from build123d import *

# Parameters (mm, degrees)
GEAR_BODY_12T_DEPTH  = 56
FACE_RECESS_SKETCH_R = 40
FACE_RECESS_80_DEPTH = 20
BORE_CUT_DEPTH       = 36


with BuildPart() as part:
    # Gear Tooth Profile Sketch → Gear Body 12T (new body)
    with BuildSketch(Plane.XY):
        with BuildLine():
            Line((-15.529142706, 57.955549577), (-17.470285544, 65.199993275))
            ThreePointArc((-17.470285544, 65.199993275), (-8.810517975, 66.922528143), (0, 67.5))
            Line((0, 67.5), (0, 60))
            ThreePointArc((0, 60), (7.831571533, 59.486691682), (15.529142706, 57.955549577))
            Line((15.529142706, 57.955549577), (17.470285544, 65.199993275))
            ThreePointArc((17.470285544, 65.199993275), (25.831131685, 62.361868445), (33.75, 58.456714755))
            Line((33.75, 58.456714755), (30, 51.961524227))
            ThreePointArc((30, 51.961524227), (36.525685741, 47.601200417), (42.426406871, 42.426406871))
            Line((42.426406871, 42.426406871), (47.72970773, 47.72970773))
            ThreePointArc((47.72970773, 47.72970773), (53.55135047, 41.091396458), (58.456714755, 33.75))
            Line((58.456714755, 33.75), (51.961524227, 30))
            ThreePointArc((51.961524227, 30), (55.432771951, 22.961005942), (57.955549577, 15.529142706))
            Line((57.955549577, 15.529142706), (65.199993275, 17.470285544))
            ThreePointArc((65.199993275, 17.470285544), (66.922528143, 8.810517975), (67.5, 0))
            Line((67.5, 0), (60, 0))
            ThreePointArc((60, 0), (59.486691682, -7.831571533), (57.955549577, -15.529142706))
            Line((57.955549577, -15.529142706), (65.199993275, -17.470285544))
            ThreePointArc((65.199993275, -17.470285544), (62.361868445, -25.831131685), (58.456714755, -33.75))
            Line((58.456714755, -33.75), (51.961524227, -30))
            ThreePointArc((51.961524227, -30), (47.601200417, -36.525685741), (42.426406871, -42.426406871))
            Line((42.426406871, -42.426406871), (47.72970773, -47.72970773))
            ThreePointArc((47.72970773, -47.72970773), (41.091396458, -53.55135047), (33.75, -58.456714755))
            Line((33.75, -58.456714755), (30, -51.961524227))
            ThreePointArc((30, -51.961524227), (22.961005942, -55.432771951), (15.529142706, -57.955549577))
            Line((15.529142706, -57.955549577), (17.470285544, -65.199993275))
            ThreePointArc((17.470285544, -65.199993275), (8.810517975, -66.922528143), (0, -67.5))
            Line((0, -67.5), (0, -60))
            ThreePointArc((0, -60), (-7.831571533, -59.486691682), (-15.529142706, -57.955549577))
            Line((-15.529142706, -57.955549577), (-17.470285544, -65.199993275))
            ThreePointArc((-17.470285544, -65.199993275), (-25.831131685, -62.361868445), (-33.75, -58.456714755))
            Line((-33.75, -58.456714755), (-30, -51.961524227))
            ThreePointArc((-30, -51.961524227), (-36.525685741, -47.601200417), (-42.426406871, -42.426406871))
            Line((-42.426406871, -42.426406871), (-47.72970773, -47.72970773))
            ThreePointArc((-47.72970773, -47.72970773), (-53.55135047, -41.091396458), (-58.456714755, -33.75))
            Line((-58.456714755, -33.75), (-51.961524227, -30))
            ThreePointArc((-51.961524227, -30), (-55.432771951, -22.961005942), (-57.955549577, -15.529142706))
            Line((-57.955549577, -15.529142706), (-65.199993275, -17.470285544))
            ThreePointArc((-65.199993275, -17.470285544), (-66.922528143, -8.810517975), (-67.5, 0))
            Line((-67.5, 0), (-60, 0))
            ThreePointArc((-60, 0), (-59.486691682, 7.831571533), (-57.955549577, 15.529142706))
            Line((-57.955549577, 15.529142706), (-65.199993275, 17.470285544))
            ThreePointArc((-65.199993275, 17.470285544), (-62.361868445, 25.831131685), (-58.456714755, 33.75))
            Line((-58.456714755, 33.75), (-51.961524227, 30))
            ThreePointArc((-51.961524227, 30), (-47.601200417, 36.525685741), (-42.426406871, 42.426406871))
            Line((-42.426406871, 42.426406871), (-47.72970773, 47.72970773))
            ThreePointArc((-47.72970773, 47.72970773), (-41.091396458, 53.55135047), (-33.75, 58.456714755))
            Line((-33.75, 58.456714755), (-30, 51.961524227))
            ThreePointArc((-30, 51.961524227), (-22.961005942, 55.432771951), (-15.529142706, 57.955549577))
        make_face()
    extrude(amount=-GEAR_BODY_12T_DEPTH)

    # Face Recess Sketch → Face Recess Ø80 (cut)
    with BuildSketch(Plane.XY):
        Circle(FACE_RECESS_SKETCH_R)
    extrude(amount=-FACE_RECESS_80_DEPTH, mode=Mode.SUBTRACT)

    # Bore Profile Sketch → Bore Cut (cut)
    with BuildSketch(Plane.XY.offset(-20)):
        with BuildLine():
            Line((0, -37), (10, -37))
            Line((10, -37), (10, -25.079872408))
            ThreePointArc((10, -25.079872408), (0, 27), (-10, -25.079872408))
            Line((-10, -25.079872408), (-10, -37))
            Line((-10, -37), (0, -37))
        make_face()
    extrude(amount=-BORE_CUT_DEPTH, mode=Mode.SUBTRACT)


solid = part.part
For this review, take the finished solid that the model builds, in its own axes (mm). A direction names the side the tool comes from. Round coordinates to 2 decimals unless told otherwise and drop trailing zeros. Write each loop counter-clockwise with the first axis right and the second up, starting at its lowest first coordinate (ties: lowest second). Pieces come first, ordered by that corner, then holes. Notation, with made-up numbers: M -34,-37.5 L -7,-37.5 A20 cw -7,-3.5 Z; hole C 75.5,-10.5 d10. An arc over 180 degrees is marked long. Write item = value, one per line. Start each with the question number.
(1) For line 1 along X through (y, z) = (-1, -29); line 2 along Y through (x, z) = (61.5, -21.5); line 3 along X through (y, z) = (34, -4), list the stretches that pass through material, from the lowest coordinate up.
(2) Clearance check with flat-ended pins moving along their axes: pin 1 Ø8 at (y, z) = (42.5, -36.5) entering from +X; pin 2 Ø12 at (x, y) = (-0.5, -19.5) entering from +Z; pin 3 Ø2 at (x, z) = (33.5, -14.5) entering from +Y; pin 4 Ø6 at (y, z) = (-33.5, -40) entering from +X. State where each tip first meets the part, or that it passes through.
(3) For faces 1 (the face through (55.25, -31.9, -27.61)), 2 (the face through (-45, 45, -28)), 3 (the face through (61.527, -16.486, -27.608)), list the 3-axis set-ups (+Z, -Z, +X, -X, +Y, -Y) from which the entire face can be reached by the end or side of a thin tool; tool diameter is ignored.
(4) We need section A-A (y = 55). Give the boundary of the cut face in (x, z), then the cut area to 3 significant figures.
(5) We need section B-B (x = 21.5). Give the boundary of the cut face in (y, z), then the cut area to 3 significant figures.
(6) The part is to be moulded in two halves that separate along X. For faces 4 (the face through (-41.189, 53.476, -27.608)), 5 (the face through (53.476, 41.189, -27.608)), 6 (the face through (-55.25, 31.9, -27.61)), say which applies: +X half, -X half, draft (parallel to the pull), parting line (faces both ways), or undercut.
Results found:
q1.line_1 = -67.49 to -26.98, 26.98 to 59.99
q1.line_2 = -27.82 to -16.48, 0 to 16.48
q1.line_3 = -49.44 to -21.07, 21.07 to 58.31
q2.pin_1 = 55.44
q2.pin_2 = through
q2.pin_3 = 59.16
q2.pin_4 = 60.22
q3.face_1 = +Z, -Z, -Y
q3.face_2 = +Z, -Z, -X
q3.face_3 = +Z, -Z, +X
q4.outline = M -39.13,-56 L -31.75,-56 L -31.75,0 L -39.13,0 Z; M -23.98,-56 L 31.75,-56 L 31.75,0 L -23.98,0 Z
q4.area = 3,530 mm²
q5.outline = M -56.02,-56 L -16.33,-56 L -16.33,-20 L -33.73,-20 L -33.73,0 L -56.02,0 Z; M 16.33,-56 L 63.98,-56 L 63.98,0 L 33.73,0 L 33.73,-20 L 16.33,-20 Z
q5.area = 4,190 mm²
q6.face_4 = -X half
q6.face_5 = +X half
q6.face_6 = undercut
